Verification items for the finished model (mm, model axes). A direction names the side the tool comes from. Coordinates: 2 decimals unless noted, no trailing zeros. Write each loop counter-clockwise with the first axis right and the second up, starting at its lowest first coordinate (ties: lowest second). Pieces come first, ordered by that corner, then holes. Notation, with made-up numbers: M 16,52 L 67,52 A34 cw 67,82 Z; hole C -33.5,-13.5 d3. An arc over 180 degrees is marked long. One line per item, written item: value.
```python
from build123d import *

# Parameters (mm, degrees)
SKETCH1_W           = 60
SKETCH1_H           = 30
BOSS_EXTRUDE1_DEPTH = 299
SKETCH2_W           = 8
SKETCH2_H           = 10
CUT_EXTRUDE1_DEPTH  = 646
CHAMFER1_SIZE       = 2


with BuildPart() as part:
    # Sketch1 → Boss-Extrude1 (new, symmetric)
    with BuildSketch(Plane.XY):
        with Locations((720, 45)):
            Rectangle(SKETCH1_W, SKETCH1_H)
    extrude(amount=BOSS_EXTRUDE1_DEPTH, both=True)

    # Sketch2 → Cut-Extrude1 (cut)
    with BuildSketch(Plane(origin=(0, 0, -299), x_dir=(-1, 0, 0), z_dir=(0, 0, -1))):
        with Locations((-735, 60)):
            Rectangle(SKETCH2_W, SKETCH2_H)
        with Locations((-750, 45)):
            Rectangle(SKETCH2_W, SKETCH2_H)
        with Locations((-690, 45)):
            Rectangle(SKETCH2_W, SKETCH2_H)
        with Locations((-705, 60)):
            Rectangle(SKETCH2_W, SKETCH2_H)
    extrude(amount=-CUT_EXTRUDE1_DEPTH, mode=Mode.SUBTRACT)

    # Chamfer1
    chamfer1_edges = [part.edges().sort_by_distance(p)[0] for p in [
        (690, 60, 0),
        (750, 60, 0),
    ]]
    chamfer(chamfer1_edges, length=CHAMFER1_SIZE)


solid = part.part
```
Item 1: Go/stop test with flat-tipped pins: P1, Ø6.5, axis at x = 735.5, z = 85, coming from the +Y side; P2, Ø3, axis at y = 44.5, z = -18, coming from the +X side; P3, Ø3, axis at y = 43, z = 26.5, coming from the -X side. Record where each tip stops, or that it passes through.
The answers:
P1: stops at y = 55
P2: stops at x = 746
P3: stops at x = 694
Item 2: Scan lines: line 1 (X direction, y = 56.5, z = 212); line 2 (Y direction, x = 701.5, z = -129.5); line 3 (X direction, y = 47.25, z = -258). Record each from-to range of solid material in increasing order.
The answers:
line 1: x = 690 to 701, 709 to 731, 739 to 750
line 2: y = 30 to 55
line 3: x = 694 to 746
Item 3: Access from +Z, -Z, +X, -X, +Y, -Y to the whole of each face (thin tool, end or side, straight path). Record for faces 1 (the face through (720, 30, 4)), 2 (the face through (746, 45, -4)).
The answers:
face 1: +Z, -Z, +X, -X, -Y
face 2: +Z, -Z, +X
Item 4: Draft check along Y on faces 3 (the face through (694, 45, -4)), 4 (the face through (690, 35, 4)), 5 (the face through (720, 60, 4)). Enter one of: released by +Y, released by -Y, zero draft, split by the parting line, or undercut.
The answers:
face 3: undercut
face 4: zero draft
face 5: released by +Y
Item 5: Cross-section at A-A, the plane z = -147.5. Enter the section's corners in (x, y).
The answers:
outline: M 690,30 L 750,30 L 750,40 L 746,40 L 746,50 L 750,50 L 750,58 L 748,60 L 739,60 L 739,55 L 731,55 L 731,60 L 709,60 L 709,55 L 701,55 L 701,60 L 692,60 L 690,58 L 690,50 L 694,50 L 694,40 L 690,40 Z
